from build123d import *

# Parameters (mm, degrees)
SKETCH1_R          = 4.188125
EXTRUDE1_DEPTH     = 8.4
SKETCH2_OUTSIDE_W  = 23.168
SKETCH2_OUTSIDE_H  = 25.644
SKETCH2_OUTSIDE_R  = 7.3
CUT_EXTRUDE2_DEPTH = 0.6
SKETCH3_OUTSIDE_W  = 78.002
SKETCH3_OUTSIDE_H  = 80.478
SKETCH3_OUTSIDE_R  = 8
CUT_EXTRUDE3_DEPTH = 15.828800806
CUT_EXTRUDE3_DRAFT = -60
CHAMFER1_SIZE      = 0.42


with BuildPart() as part:
    # Sketch1 → Extrude1 (new body)
    with BuildSketch(Plane.XY):
        Polygon((0, 9.237604307), (-8, 4.618802154), (-8, -4.618802154), (0, -9.237604307), (8, -4.618802154), (8, 4.618802154), align=None)
        Circle(SKETCH1_R, mode=Mode.SUBTRACT)
    extrude(amount=EXTRUDE1_DEPTH)

    # Sketch2 outside → Cut-Extrude2 (cut)
    with BuildSketch(Plane.XY):
        Rectangle(SKETCH2_OUTSIDE_W, SKETCH2_OUTSIDE_H)
        Circle(SKETCH2_OUTSIDE_R, mode=Mode.SUBTRACT)
    extrude(amount=CUT_EXTRUDE2_DEPTH, mode=Mode.SUBTRACT)


with BuildPart() as cut_extrude3_tool:
    # Sketch3 outside → Cut-Extrude3 (with draft: the straight prism first)
    with BuildSketch(Plane.XY.offset(8.4)):
        Rectangle(SKETCH3_OUTSIDE_W, SKETCH3_OUTSIDE_H)
        Circle(SKETCH3_OUTSIDE_R, mode=Mode.SUBTRACT)
    extrude(amount=-CUT_EXTRUDE3_DEPTH)
    # Cut-Extrude3: the draft: its side faces are tilted about the plane it starts from
    cut_extrude3_sides = [cut_extrude3_tool.faces().sort_by_distance(p)[0] for p in [
        (0, -40.239, 0.485599597),
        (39.001, 0, 0.485599597),
        (0, 40.239, 0.485599597),
        (-39.001, 0, 0.485599597),
        (-8, 0, 0.485599597),
    ]]
    draft(cut_extrude3_sides, Plane.XY.offset(8.4), CUT_EXTRUDE3_DRAFT)


with BuildPart() as part_1:
    add(part.part)

    # Cut-Extrude3: cut by cut_extrude3_tool
    add(cut_extrude3_tool.part, mode=Mode.SUBTRACT)

    # Chamfer1
    chamfer1_edges = [part_1.edges().sort_by_distance(p)[0] for p in [
        (-4.188125, 0, 0),
        (-4.188125, 0, 8.4),
    ]]
    chamfer(chamfer1_edges, length=CHAMFER1_SIZE)


solid = part_1.part
Source: CAD feature listing. Evaluate the final solid. Frame: model axes, mm. A direction names the side the tool comes from. Give positions to 0.01 mm unless a question says otherwise; leave off trailing zeros. Write each loop counter-clockwise with the first axis right and the second up, starting at its lowest first coordinate (ties: lowest second). Pieces come first, ordered by that corner, then holes. Notation, with made-up numbers: (25.25, 0.5) -> (49.25, 0.5) arc R22 ccw to (49.25, 18.5) -> close; hole circle Ø9 at (33.25, -30.75). An arc over 180 degrees is marked (long way). Return JSON: item names as keys, results as strings. Group by question number.
1. Section A-A, the plane z = 3. Output: boundary loops of the cut face in (x, y).
2. Material intervals for line 1 (X direction, y = 3.5, z = 1.75); line 2 (Y direction, x = 2.25, z = 7); line 3 (X direction, y = -0.5, z = 6), sorted ascending. Write a range as from..to.
3. Access query for faces 4 (the face through (6.963, 2.193, 0.296)), 5 (the face through (7.17, -4.17, 8.23)). Directions: +Z, -Z, +X, -X, +Y, -Y. A direction counts if a zero-diameter tool reaches every point of the face in a straight line with its end or side. Return the directions, or none.
4. Mould query, pull axis X, two halves, no side actions, for faces 1 (the face through (0, -5, 0)), 2 (the face through (4.056, 6.896, 4.445)), 3 (the face through (-3.09, 2.83, 4.15)). Classes: +X half, -X half, draft (parallel to the pull), parting line (faces both ways), or undercut.
5. Pin query (flat end, axial travel): pin 1 Ø7.5 at (x, y) = (0, 0) entering from +Z. Return the tip coordinate at first contact, or that it passes through.
Determined:
{
 "1": {"outline": "(-8, -4.62) -> (0, -9.24) -> (8, -4.62) -> (8, 4.62) -> (0, 9.24) -> (-8, 4.62) -> close; hole circle Ø8.38 at (0, 0)"},
 "2": {"line 1": "x = -8..-2.3, 2.3..8", "line 2": "y = -7.94..-3.53, 3.53..7.94", "line 3": "x = -8..-4.16, 4.16..8"},
 "3": {"face 4": "-Z", "face 5": "+Z, +X, -Y"},
 "4": {"face 1": "draft", "face 2": "+X half", "face 3": "undercut"},
 "5": {"pin 1": "passes through"}
}
